Read the model definition and answer for the solid it produces. Units are mm, in the model's axes. Coordinates: 2 decimals unless noted, no trailing zeros. Write each loop counter-clockwise with the first axis right and the second up, starting at its lowest first coordinate (ties: lowest second). Pieces come first, ordered by that corner, then holes. Notation, with made-up numbers: (44.25, 72.25) -> (56.25, 72.25) arc R26 ccw to (56.25, 106.25) -> close; hole circle Ø7 at (68, 10.25). An arc over 180 degrees is marked (long way). One line per item, written item: value. Start each with the question number.
from build123d import *

# Parameters (mm, degrees)
SKETCH_1_W             = 930
SKETCH_1_H             = 60
EXTRUDE_1_DEPTH        = 30
PATTERN_LINEAR_1_COUNT = 6
PATTERN_LINEAR_1_PITCH = 140


with BuildPart() as part:
    # 草图1 → 凸台-拉伸1 (new body)
    with BuildSketch(Plane(origin=(0, 0, 0), x_dir=(1, 0, 0), z_dir=(0, 1, 0))):
        Rectangle(SKETCH_1_W, SKETCH_1_H)
    extrude(amount=EXTRUDE_1_DEPTH)

    # 草图3 → 切除-旋转1 (revolve, cut)
    with BuildSketch(Plane.XY, mode=Mode.PRIVATE) as cut_revolve_1_sk:
        Polygon((350, 30), (375, 30), (375, 25), (370, 25), (370, 0), (350, 0), align=None)
    cut_revolve_1 = revolve(cut_revolve_1_sk.sketch.rotate(Axis((350, 0, 0), (0, 1, 0)), 90), axis=Axis((350, 0, 0), (0, 1, 0)), mode=Mode.SUBTRACT)

    # 阵列(线性)1: 切除-旋转1 ×6
    with Locations(*[(-i * PATTERN_LINEAR_1_PITCH, 0, 0) for i in range(1, PATTERN_LINEAR_1_COUNT)]):
        add(cut_revolve_1, mode=Mode.SUBTRACT)


solid = part.part
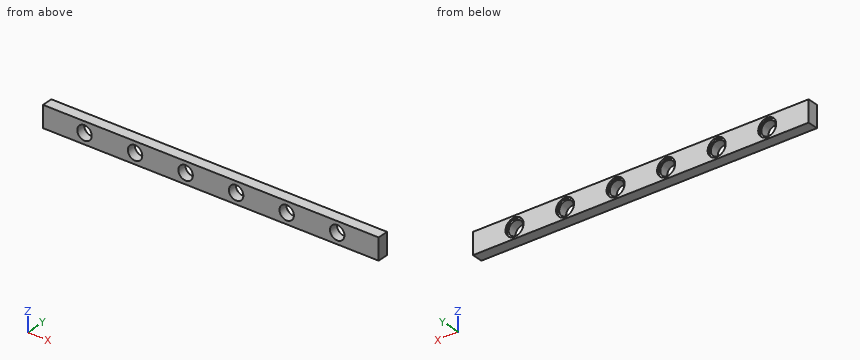
1. A cutting plane is placed at A-A on x = 70. Give the vertices of the cut face in (y, z), then the cut area to 3 significant figures.
2. Find the intervals of material crossed by probe 1 along Z at (x, y) = (-210, 26.9); probe 2 along Z at (x, y) = (350, 6.75); probe 3 along Y at (x, z) = (330, -4.5), in increasing order. Write a range as from..to.
3. A cutting plane is placed at B-B on y = 13.75. Give the vertices of the cut face in (x, z).
4. A cutting plane is placed at C-C on z = 0. Count the separate pieces of the cut face and the enclosed holes in it, then the cut area to 3 significant figures.
Derived:
1. outline: (0, -30) -> (30, -30) -> (30, -25) -> (25, -25) -> (25, -20) -> (0, -20) -> close; (0, 20) -> (25, 20) -> (25, 25) -> (30, 25) -> (30, 30) -> (0, 30) -> close
1. area: 550 mm2
2. probe 1: z = -30..-25, 25..30
2. probe 2: z = -30..-20, 20..30
2. probe 3: y = 0..25
3. outline: (-465, -30) -> (465, -30) -> (465, 30) -> (-465, 30) -> close; hole circle Ø40 at (-350, 0); hole circle Ø40 at (-210, 0); hole circle Ø40 at (-70, 0); hole circle Ø40 at (70, 0); hole circle Ø40 at (210, 0); hole circle Ø40 at (350, 0)
4. separate pieces: 7
4. enclosed holes: 0
4. area: 20,400 mm2
